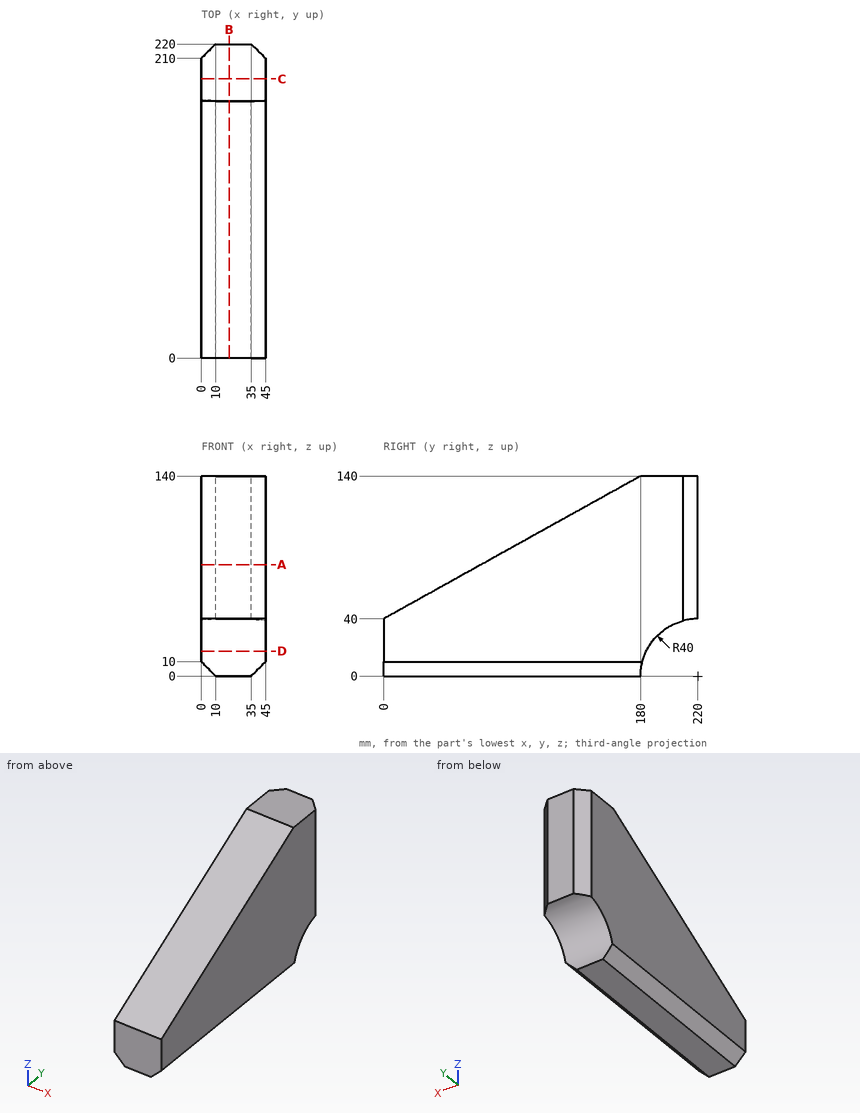
Check sheet for the drawn part. Datum: minimum x, y, z corner. Units: mm. Round coordinates to 2 decimals unless told otherwise and drop trailing zeros. Order: outer loops, then holes, each group sorted by start corner. A loop starts at its lowest first (then second) coordinate and runs counter-clockwise, first axis right, second up.
1) Scan lines: line 1 (Y direction, x = 27.5, z = 66.5); line 2 (Y direction, x = 38, z = 53.5); line 3 (Z direction, x = 4, y = 196). Record each from-to range of solid material in increasing order.
2) Section check C-C (y = 195.5). Record the boundary of the cut face in (x, z).
3) Section check B-B (x = 19.5). Record the boundary of the cut face in (y, z), and give its area (3 significant figures).
4) Section check A-A (z = 78). Record the boundary of the cut face in (x, y).
5) Go/stop test with flat-tipped pins: pin 1 Ø12 at (x, z) = (39, 58.5) entering from -Y; pin 2 Ø6 at (x, z) = (36, 64) entering from -Y. Record where each tip stops, or that it passes through.
6) Section check D-D (z = 17.5). Record the boundary of the cut face in (x, y), and give its area (3 significant figures).
Result:
1. line 1: y = 47.7 to 220
1. line 2: y = 24.3 to 217
1. line 3: z = 32 to 140
2. outline: (0, 31.62) - (45, 31.62) - (45, 140) - (0, 140) - close
3. outline: (0, 0) - (180, 0) arc R40 cw to (220, 40) - (220, 140) - (180, 140) - (0, 40) - close
3. area: 20,500 mm2
4. outline: (0, 68.4) - (45, 68.4) - (45, 210) - (35, 220) - (10, 220) - (0, 210) - close
5. pin 1: stops at y = 22.5
5. pin 2: stops at y = 37.8
6. outline: (0, 0) - (45, 0) - (45, 184.03) - (0, 184.03) - close
6. area: 8,280 mm2
